Verification items for the finished model (mm, model axes). Coordinates: 2 decimals unless noted, no trailing zeros. Order: outer loops, then holes, each group sorted by start corner. A loop starts at its lowest first (then second) coordinate and runs counter-clockwise, first axis right, second up. Notation, with made-up numbers: M -36.75,8.5 L 1.25,8.5 A20 ccw 1.25,22.5 Z; hole C -10.5,67 d11. An arc over 180 degrees is marked long. Return JSON: item names as keys, results as strings.
```python
from build123d import *

# Parameters (mm, degrees)
SKETCH_3_R          = 3.3234375
EXTRUDE_1_DEPTH     = 6.8
SKETCH_5_R          = 10.785
SKETCH_5_R_2        = 6.5
CUT_EXTRUDE_1_DEPTH = 1.36
CUT_EXTRUDE_1_DRAFT = -60
SKETCH_7_R          = 10.785
SKETCH_7_R_2        = 6.5
CUT_EXTRUDE_2_DEPTH = 1.36
CUT_EXTRUDE_2_DRAFT = -60


with BuildPart() as part:
    # 草图3 → 凸台-拉伸1 (new body)
    with BuildSketch(Plane.XY):
        Polygon((0, 7.505553499), (-6.5, 3.75277675), (-6.5, -3.75277675), (0, -7.505553499), (6.5, -3.75277675), (6.5, 3.75277675), align=None)
        Circle(SKETCH_3_R, mode=Mode.SUBTRACT)
    extrude(amount=-EXTRUDE_1_DEPTH)

    # 草图4 → 切除-旋转1 (revolve, cut)
    with BuildSketch(Plane(origin=(0, 0, 0), x_dir=(0, 0, -1), z_dir=(1, 0, 0)), mode=Mode.PRIVATE) as cut_revolve_1_sk:
        Polygon((0, 4.375), (0.607119892, 3.3234375), (0.607119892, 0), (0, 0), align=None)
        Polygon((6.8, 0), (6.8, 4.375), (6.192880108, 3.3234375), (6.192880108, 0), align=None)
    revolve(cut_revolve_1_sk.sketch.rotate(Axis((0, 0, 0), (0, 0, -1)), 90), axis=Axis((0, 0, 0), (0, 0, -1)), mode=Mode.SUBTRACT)


with BuildPart() as cut_extrude_1_tool:
    # 草图5 → 切除-拉伸1 (with draft: the straight prism first)
    with BuildSketch(Plane.XY):
        Circle(SKETCH_5_R)
        Circle(SKETCH_5_R_2, mode=Mode.SUBTRACT)
    extrude(amount=-CUT_EXTRUDE_1_DEPTH)
    # 切除-拉伸1: the draft: its side faces are tilted about the plane it starts from
    cut_extrude_1_sides = [cut_extrude_1_tool.faces().sort_by_distance(p)[0] for p in [
        (-10.785, 0, -0.68),
        (-6.5, 0, -0.68),
    ]]
    draft(cut_extrude_1_sides, Plane.XY, CUT_EXTRUDE_1_DRAFT)


with BuildPart() as part_1:
    add(part.part)

    # 切除-拉伸1: cut by cut_extrude_1_tool
    add(cut_extrude_1_tool.part, mode=Mode.SUBTRACT)


with BuildPart() as cut_extrude_2_tool:
    # 草图7 → 切除-拉伸2 (with draft: the straight prism first)
    with BuildSketch(Plane(origin=(0, 0, -6.8), x_dir=(-1, 0, 0), z_dir=(0, 0, -1))):
        Circle(SKETCH_7_R)
        Circle(SKETCH_7_R_2, mode=Mode.SUBTRACT)
    extrude(amount=-CUT_EXTRUDE_2_DEPTH)
    # 切除-拉伸2: the draft: its side faces are tilted about the plane it starts from
    cut_extrude_2_sides = [cut_extrude_2_tool.faces().sort_by_distance(p)[0] for p in [
        (10.785, 0, -6.12),
        (6.5, 0, -6.12),
    ]]
    draft(cut_extrude_2_sides, Plane(origin=(0, 0, -6.8), x_dir=(-1, 0, 0), z_dir=(0, 0, -1)), CUT_EXTRUDE_2_DRAFT)


with BuildPart() as part_2:
    add(part_1.part)

    # 切除-拉伸2: cut by cut_extrude_2_tool
    add(cut_extrude_2_tool.part, mode=Mode.SUBTRACT)


solid = part_2.part
```
Q1. Material ranges on line 1 along X through (y, z) = (1, -2.75); line 2 along X through (y, z) = (0.25, -5.5); line 3 along Y through (x, z) = (1.5, -6.5), recorded low to high.
Values:
{"line 1": "-6.5 to -3.17, 3.17 to 6.5", "line 2": "-6.5 to -3.31, 3.31 to 6.5", "line 3": "-6.64 to -3.55, 3.55 to 6.64"}
Q2. Cross-section at A-A, the plane z = -2.25. Record the boundary of the cut face in (x, y), and give its area (3 significant figures).
Values:
{"outline": "M -6.5,-3.75 L 0,-7.51 L 6.5,-3.75 L 6.5,3.75 L 0,7.51 L -6.5,3.75 Z; hole C 0,0 d6.65", "area": "112 mm^2"}
Q3. Go/stop test with flat-tipped pins: pin 1 (1 mm diameter, centred on x = -1, y = 2, fed in from +Z); pin 2 (1.5 mm diameter, centred on y = 5, z = -3.5, fed in from +X). Record where each tip stops, or that it passes through.
Values:
{"pin 1": "through", "pin 2": "x = 5.64"}
Q4. Draft check along X on faces 1 (the face through (5.845, 3.356, -0.138)), 2 (the face through (0.02, 6.74, -0.14)), 3 (the face through (-2.64, -2.02, -3.36)), 4 (the face through (-5.83, -3.38, -6.66)). Enter one of: pulls with the +X half, pulls with the -X half, needs draft (parallel to the pull), parting line crosses it, or undercut.
Values:
{"face 1": "pulls with the +X half", "face 2": "parting line crosses it", "face 3": "undercut", "face 4": "pulls with the -X half"}
